```python
from build123d import *

# Parameters (mm, degrees)
WHEEL_DISC_SKETCH_R        = 125
WHEEL_DISC_250_DEPTH       = 78
FACE_RECESS_SKETCH_R       = 97.533404225
FACE_RECESS_SKETCH_R_2     = 81.367148925
FACE_RECESS_5MM_DEPTH      = 5
LIGHTENING_HOLE_1_SKETCH_R = 19.5
LIGHTENING_HOLE_1_39_DEPTH = 78
LIGHTENING_HOLE_2_SKETCH_R = 19.5
LIGHTENING_HOLE_2_39_DEPTH = 78
LIGHTENING_HOLE_3_SKETCH_R = 19.5
LIGHTENING_HOLE_3_39_DEPTH = 78
LIGHTENING_HOLE_4_SKETCH_R = 19.5
LIGHTENING_HOLE_4_39_DEPTH = 78
HUB_BOSS_SKETCH_R          = 25
HUB_BOSS_SKETCH_R_2        = 12.5
HUB_BOSS_50_DEPTH          = 16
CENTRE_START               = -78
CENTRE_CUT_SKETCH_R        = 12.5
CENTRE_CUT_DEPTH           = 78


with BuildPart() as part:
    # Wheel Disc Sketch → Wheel Disc Ø250 (new body)
    with BuildSketch(Plane.XY):
        Circle(WHEEL_DISC_SKETCH_R)
    extrude(amount=-WHEEL_DISC_250_DEPTH)

    # Face Recess Sketch → Face Recess 5mm (cut)
    with BuildSketch(Plane.XY):
        Circle(FACE_RECESS_SKETCH_R)
        Circle(FACE_RECESS_SKETCH_R_2, mode=Mode.SUBTRACT)
    extrude(amount=-FACE_RECESS_5MM_DEPTH, mode=Mode.SUBTRACT)

    # Lightening Hole 1 Sketch → Lightening Hole 1 Ø39 (cut)
    with BuildSketch(Plane.XY):
        with Locations((0, 49.162629863)):
            Circle(LIGHTENING_HOLE_1_SKETCH_R)
    extrude(amount=-LIGHTENING_HOLE_1_39_DEPTH, mode=Mode.SUBTRACT)

    # Lightening Hole 2 Sketch → Lightening Hole 2 Ø39 (cut)
    with BuildSketch(Plane.XY):
        with Locations((49.162629863, 0)):
            Circle(LIGHTENING_HOLE_2_SKETCH_R)
    extrude(amount=-LIGHTENING_HOLE_2_39_DEPTH, mode=Mode.SUBTRACT)

    # Lightening Hole 3 Sketch → Lightening Hole 3 Ø39 (cut)
    with BuildSketch(Plane.XY):
        with Locations((0, -49.162629863)):
            Circle(LIGHTENING_HOLE_3_SKETCH_R)
    extrude(amount=-LIGHTENING_HOLE_3_39_DEPTH, mode=Mode.SUBTRACT)

    # Lightening Hole 4 Sketch → Lightening Hole 4 Ø39 (cut)
    with BuildSketch(Plane.XY):
        with Locations((-49.162629863, 0)):
            Circle(LIGHTENING_HOLE_4_SKETCH_R)
    extrude(amount=-LIGHTENING_HOLE_4_39_DEPTH, mode=Mode.SUBTRACT)

    # Hub Boss Sketch → Hub Boss Ø50 (add)
    with BuildSketch(Plane.XY.offset(-5)):
        Circle(HUB_BOSS_SKETCH_R)
        Circle(HUB_BOSS_SKETCH_R_2, mode=Mode.SUBTRACT)
    extrude(amount=HUB_BOSS_50_DEPTH)

    # Centre Cut Sketch → Centre Cut (cut)
    with BuildSketch(Plane.XY.offset(CENTRE_START)):
        Circle(CENTRE_CUT_SKETCH_R)
    extrude(amount=CENTRE_CUT_DEPTH, mode=Mode.SUBTRACT)


solid = part.part
```
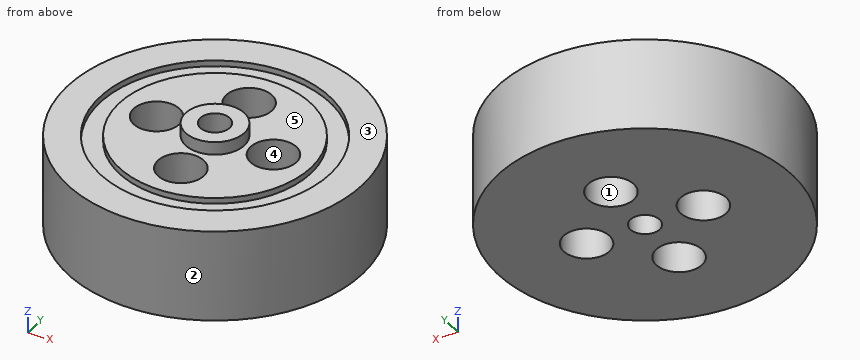
The model under review builds one solid part; all positions refer to its coordinate system, in mm. Face numbers are marked on the shaded views. A direction names the side the tool comes from. Round coordinates to 2 decimals unless told otherwise and drop trailing zeros. Loops run counter-clockwise (first coordinate to the right, second up) from the corner with the lowest first, then second, coordinate; pieces in that order, holes last. Notation, with made-up numbers: M 76.5,10.25 L 132.5,10.25 A16 ccw 132.5,37.25 Z; hole C 86,-27.5 d11. An arc over 180 degrees is marked long. Put each result on its own line as item: value.
Q1. For pin 1 (12 mm diameter, centred on x = 76.5, z = -38.5, fed in from -Y); pin 2 (4 mm diameter, centred on y = -98.5, z = -67.5, fed in from +X); pin 3 (3 mm diameter, centred on x = 47.5, z = -11, fed in from +Y); pin 4 (20 mm diameter, centred on x = 0, y = 0, fed in from +Z), all flat-tipped, find the tip position at first contact; note any pin that passes through.
Result set:
pin 1: stops at y = -103.22
pin 2: stops at x = 79.45
pin 3: stops at y = 116.23
pin 4: passes through
Q2. To check wall thickness, follow L1, parallel to Y at x = 0, z = -36; L2, parallel to Y at x = 0, z = -2.7; L3, parallel to X at y = 37.5, z = -3.5. State the ranges of each line that lie inside material, in increasing order.
Result set:
L1: y = -125 to -68.66, -29.66 to -12.5, 12.5 to 29.66, 68.66 to 125
L2: y = -125 to -97.53, -81.37 to -68.66, -29.66 to -12.5, 12.5 to 29.66, 68.66 to 81.37, 97.53 to 125
L3: x = -119.24 to -90.04, -72.21 to -15.63, 15.63 to 72.21, 90.04 to 119.24
Q3. Machinability: for the marked faces 4 and 5, which of the approach directions +Z, -Z, +X, -X, +Y, -Y give a long, thin tool a straight path to every point of the face, cutting with its end or side? Answer none if there is none.
Result set:
face 4: +Z, -Z
face 5: +Z
Q4. Consider section A-A, the plane x = 0. Give the boundary of the cut face in (y, z), then the cut area to 3 significant figures.
Result set:
outline: M -125,-78 L -68.66,-78 L -68.66,0 L -81.37,0 L -81.37,-5 L -97.53,-5 L -97.53,0 L -125,0 Z; M -29.66,-78 L -12.5,-78 L -12.5,11 L -25,11 L -25,0 L -29.66,0 Z; M 12.5,-78 L 29.66,-78 L 29.66,0 L 25,0 L 25,11 L 12.5,11 Z; M 68.66,-78 L 125,-78 L 125,0 L 97.53,0 L 97.53,-5 L 81.37,-5 L 81.37,0 L 68.66,0 Z
area: 11,600 mm²
Q5. Consider section D-D, the plane x = -87. Give the boundary of the cut face in (y, z).
Result set:
outline: M -89.76,-78 L 89.76,-78 L 89.76,0 L 44.09,0 L 44.09,-5 L -44.09,-5 L -44.09,0 L -89.76,0 Z
Q6. Consider section C-C, the plane y = -57.5. Give the boundary of the cut face in (x, z).
Result set:
outline: M -110.99,-78 L -17.63,-78 L -17.63,0 L -57.57,0 L -57.57,-5 L -78.78,-5 L -78.78,0 L -110.99,0 Z; M 17.63,-78 L 110.99,-78 L 110.99,0 L 78.78,0 L 78.78,-5 L 57.57,-5 L 57.57,0 L 17.63,0 Z
Q7. Mouldability with a two-part tool opening along Y and no side actions: class the marked faces 1, 2 and 3 as released by +Y, released by -Y, zero draft, split by the parting line, or undercut.
Result set:
face 1: undercut
face 2: split by the parting line
face 3: zero draft
